Geometry: see drawing. Coordinates: mm, zero at the bounding-box minimum. Round coordinates to 2 decimals unless told otherwise and drop trailing zeros. Loops run counter-clockwise (first coordinate to the right, second up) from the corner with the lowest first, then second, coordinate; pieces in that order, holes last.
(1) Cut plane C-C, the plane x = 72. Output: boundary loops of the cut face in (y, z), and give its area (3 significant figures).
(2) Cut plane D-D, the plane y = 7. Output: boundary loops of the cut face in (x, z), and give its area (3 significant figures).
(3) Line query: line 1 (Y direction, x = 20, z = 12.5); line 2 (Y direction, x = 132, z = 8.5); line 3 (X direction, y = 32, z = 11.75). Output: solid intervals per line, ascending.
(4) Cut plane B-B, the plane z = 8.5. Output: boundary loops of the cut face in (x, y).
(5) Cut plane A-A, the plane x = 20. Output: boundary loops of the cut face in (y, z).
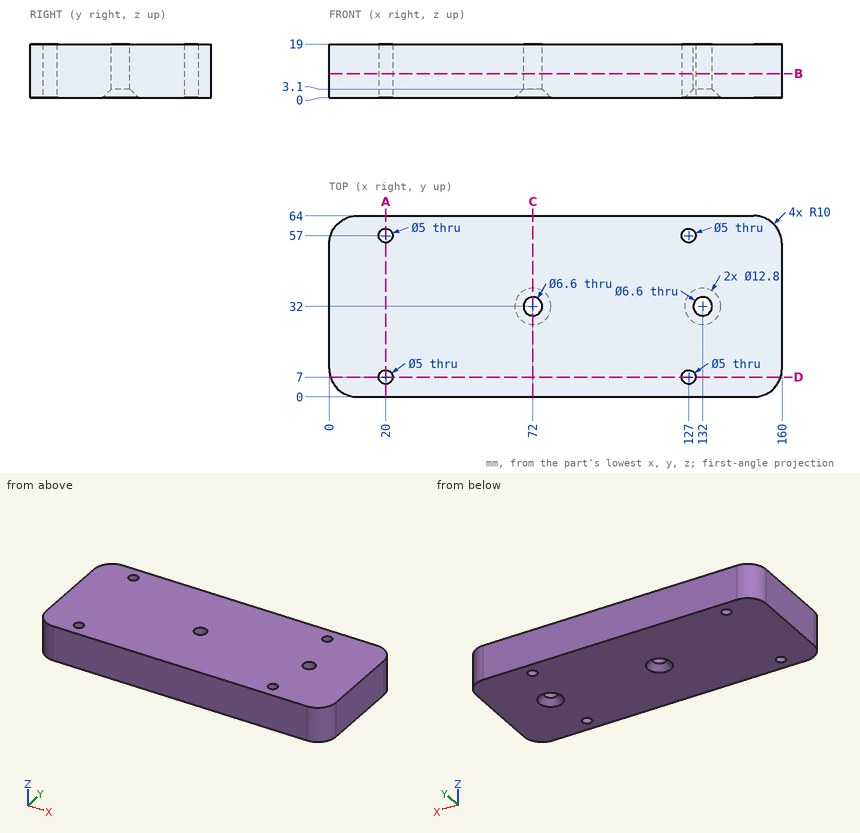
Reported:
1. outline: (0, 0) - (25.6, 0) - (28.7, 3.1) - (28.7, 19) - (0, 19) - close; (35.3, 3.1) - (38.4, 0) - (64, 0) - (64, 19) - (35.3, 19) - close
1. area: 1,080 mm2
2. outline: (0.46, 0) - (17.5, 0) - (17.5, 19) - (0.46, 19) - close; (22.5, 0) - (124.5, 0) - (124.5, 19) - (22.5, 19) - close; (129.5, 0) - (159.54, 0) - (159.54, 19) - (129.5, 19) - close
2. area: 2,830 mm2
3. line 1: y = 0 to 4.5, 9.5 to 54.5, 59.5 to 64
3. line 2: y = 0 to 28.7, 35.3 to 64
3. line 3: x = 0 to 68.7, 75.3 to 128.7, 135.3 to 160
4. outline: (0, 10) arc R10 ccw to (10, 0) - (150, 0) arc R10 ccw to (160, 10) - (160, 54) arc R10 ccw to (150, 64) - (10, 64) arc R10 ccw to (0, 54) - close; hole circle Ø5 at (20, 7); hole circle Ø5 at (20, 57); hole circle Ø6.6 at (72, 32); hole circle Ø5 at (127, 7); hole circle Ø5 at (127, 57); hole circle Ø6.6 at (132, 32)
5. outline: (0, 0) - (4.5, 0) - (4.5, 19) - (0, 19) - close; (9.5, 0) - (54.5, 0) - (54.5, 19) - (9.5, 19) - close; (59.5, 0) - (64, 0) - (64, 19) - (59.5, 19) - close
